from build123d import *

# Parameters (mm, degrees)
BOSS_EXTRUDE2_DEPTH   = 7
M6_TAPPED_HOLE1_D     = 5
M6_TAPPED_HOLE1_DEPTH = 15
M6_TAPPED_HOLE1_TIP   = 1.502151548
M6_TAPPED_HOLE2_D     = 5
M6_TAPPED_HOLE2_DEPTH = 15
M6_TAPPED_HOLE2_TIP   = 1.502151548
CHAMFER1_SIZE         = 1


with BuildPart() as part:
    # Sketch6 → Boss-Extrude2 (new, symmetric)
    with BuildSketch(Plane.XY):
        Polygon((0, 0), (0, 55), (-15, 55), (-25, 25), (-25, 0), align=None)
    extrude(amount=BOSS_EXTRUDE2_DEPTH, both=True)

    # M6 Tapped Hole1
    with Locations(Plane(origin=(0, 0, 0), x_dir=(0, 0, -1), z_dir=(1, 0, 0))):
        with Locations((0, 25), (0, 47)):
            Hole(M6_TAPPED_HOLE1_D / 2, depth=M6_TAPPED_HOLE1_DEPTH)
            with Locations((0, 0, -(M6_TAPPED_HOLE1_DEPTH + M6_TAPPED_HOLE1_TIP / 2))):  # 118° drill point
                Cone(0, M6_TAPPED_HOLE1_D / 2, M6_TAPPED_HOLE1_TIP, mode=Mode.SUBTRACT)

    # M6 Tapped Hole2
    with Locations(Plane(origin=(0, 0, 0), x_dir=(-1, 0, 0), z_dir=(0, -1, 0))):
        with Locations((16, 0)):
            Hole(M6_TAPPED_HOLE2_D / 2, depth=M6_TAPPED_HOLE2_DEPTH)
            with Locations((0, 0, -(M6_TAPPED_HOLE2_DEPTH + M6_TAPPED_HOLE2_TIP / 2))):  # 118° drill point
                Cone(0, M6_TAPPED_HOLE2_D / 2, M6_TAPPED_HOLE2_TIP, mode=Mode.SUBTRACT)

    # Chamfer1
    chamfer1_edges = [part.edges().sort_by_distance(p)[0] for p in [
        (-25, 0, 0),
        (0, 55, 0),
        (0, 0, 0),
    ]]
    chamfer(chamfer1_edges, length=CHAMFER1_SIZE)


solid = part.part
Input: part model. Units: mm. Frame: model coordinates. A direction names the side the tool comes from. Coordinates: 2 decimals unless noted, no trailing zeros. Write each loop counter-clockwise with the first axis right and the second up, starting at its lowest first coordinate (ties: lowest second). Pieces come first, ordered by that corner, then holes. Notation, with made-up numbers: M 46.5,32 L 100.5,32 A23 ccw 100.5,68 Z; hole C 0,20 d9. An arc over 180 degrees is marked long. Answer as a JSON object with one key per item and string values. Group by question number.
(1) Contact query for flat-ended pins moving along their axis: P1, Ø4, axis at y = 25, z = 0, coming from the +X side; P2, Ø8, axis at y = 41.5, z = 0.5, coming from the -X side; P3, Ø2, axis at y = 36.5, z = 1.5, coming from the -X side. Output: stop coordinate, or through.
(2) Mould query, pull axis Y, two halves, no side actions, for faces 4 (the face through (-0.5, 0.5, 0.1)), 5 (the face through (-16.24, 24.83, -0.4)), 6 (the face through (0, 27, 2)), 7 (the face through (-7.6, 44.56, -0.54)). Classes: pulls with the +Y half, pulls with the -Y half, needs draft (parallel to the pull), parting line crosses it, or undercut.
(3) Section B-B on x = -8.25. Output: boundary loops of the cut face in (y, z).
(4) Section A-A on z = 5. Output: boundary loops of the cut face in (x, y).
(5) Ray query, line 1 along Y through (x, z) = (-9.75, 0); line 2 along Z through (x, y) = (-5.5, 47); line 3 along Y through (x, z) = (-9.75, -1.25). Return the intervals inside material, ascending. Write a range as [from, to].
(6) Set-up query: faces 1 (the face through (-25, 13, 0)), 2 (the face through (-7.6, 27.48, -0.33)), 3 (the face through (-18.5, 7.6, -0.1)). Return all of +Z, -Z, +X, -X, +Y, -Y with unobstructed straight access to the full face (end or side cutting, diameter ignored); none if empty.
Result set:
{
 "1": {"P1": "stops at x = -15.3", "P2": "stops at x = -20.83", "P3": "stops at x = -21.5"},
 "2": {"face 4": "pulls with the -Y half", "face 5": "undercut", "face 6": "needs draft", "face 7": "undercut"},
 "3": {"outline": "M 0,-7 L 55,-7 L 55,7 L 0,7 Z; hole C 25,0 d5; hole C 47,0 d5"},
 "4": {"outline": "M -25,1 L -24,0 L -1,0 L 0,1 L 0,54 L -1,55 L -15,55 L -25,25 Z"},
 "5": {"line 1": "y = [0, 22.5], [27.5, 44.5], [49.5, 55]", "line 2": "z = [-7, -2.5], [2.5, 7]", "line 3": "y = [0, 22.83], [27.17, 44.83], [49.17, 55]"},
 "6": {"face 1": "+Z, -Z, -X, +Y, -Y", "face 2": "+X", "face 3": "-Y"}
}
